from build123d import *

# Parameters (mm, degrees)
BASE_PLATE_140X70X20_DEPTH   = 20
CENTRE_HOLE_SKETCH_R         = 10
CENTRE_HOLE_20_DEPTH         = 20
CENTRE_POCKET_SKETCH_W       = 40
CENTRE_POCKET_SKETCH_H       = 40
CENTRE_POCKET_40X40X10_DEPTH = 10
V_BLOCK_UPRIGHTS_DEPTH       = 70
GUSSET_RIB_DEPTH             = 5


with BuildPart() as part:
    # Base Plate Sketch → Base Plate 140x70x20 (new body)
    with BuildSketch(Plane(origin=(0, 0, 0), x_dir=(1, 0, 0), z_dir=(0, 1, 0))):
        with BuildLine():
            Line((-70, 25), (-62.5, 25))
            ThreePointArc((-62.5, 25), (-57.5, 20), (-62.5, 15))
            Line((-62.5, 15), (-70, 15))
            Line((-70, 15), (-70, -15))
            Line((-70, -15), (-62.5, -15))
            ThreePointArc((-62.5, -15), (-57.5, -20), (-62.5, -25))
            Line((-62.5, -25), (-70, -25))
            Line((-70, -25), (-70, -35))
            Line((-70, -35), (70, -35))
            Line((70, -35), (70, -25))
            Line((70, -25), (62.5, -25))
            ThreePointArc((62.5, -25), (57.5, -20), (62.5, -15))
            Line((62.5, -15), (70, -15))
            Line((70, -15), (70, 15))
            Line((70, 15), (62.5, 15))
            ThreePointArc((62.5, 15), (57.5, 20), (62.5, 25))
            Line((62.5, 25), (70, 25))
            Line((70, 25), (70, 35))
            Line((70, 35), (-70, 35))
            Line((-70, 35), (-70, 25))
        make_face()
    extrude(amount=BASE_PLATE_140X70X20_DEPTH)

    # Centre Hole Sketch → Centre Hole Ø20 (cut)
    with BuildSketch(Plane(origin=(0, 20, 0), x_dir=(1, 0, 0), z_dir=(0, 1, 0))):
        with Locations(Location((0, 0, 0), (0, 0, 270))):
            Circle(CENTRE_HOLE_SKETCH_R)
    extrude(amount=-CENTRE_HOLE_20_DEPTH, mode=Mode.SUBTRACT)

    # Centre Pocket Sketch → Centre Pocket 40x40x10 (cut)
    with BuildSketch(Plane(origin=(0, 20, 0), x_dir=(1, 0, 0), z_dir=(0, 1, 0))):
        Rectangle(CENTRE_POCKET_SKETCH_W, CENTRE_POCKET_SKETCH_H)
    extrude(amount=-CENTRE_POCKET_40X40X10_DEPTH, mode=Mode.SUBTRACT)

    # V-Block Uprights Sketch → V-Block Uprights (add)
    with BuildSketch(Plane.XY.offset(35)):
        Polygon((-40, 60), (-52.5, 20), (-35, 20), (-35, 60), align=None)
        Polygon((35, 60), (35, 20), (52.5, 20), (40, 60), align=None)
    extrude(amount=-V_BLOCK_UPRIGHTS_DEPTH)

    # Gusset Rib Sketch → Gusset Rib (add, symmetric)
    with BuildSketch(Plane.XY):
        Polygon((-20.102951906, 20), (-35, 20), (-35, 52), align=None)
        Polygon((20.1, 20), (35, 52), (35, 20), align=None)
    extrude(amount=GUSSET_RIB_DEPTH, both=True)


solid = part.part
The listing builds one solid part. Answer for the finished solid, in the listing's coordinates (mm). A direction names the side the tool comes from. Round coordinates to 2 decimals unless told otherwise and drop trailing zeros. Order: outer loops, then holes, each group sorted by start corner. A loop starts at its lowest first (then second) coordinate and runs counter-clockwise, first axis right, second up. Notation, with made-up numbers: M 1.25,21.5 L 49.25,21.5 A8 ccw 49.25,28.5 Z; hole C -22,-35.5 d4. An arc over 180 degrees is marked long. Answer in a Markdown table with one row per item. Add a question column.
1) Flat-ended cylindrical pins translate along their axes: pin 1 Ø1 at (y, z) = (53.5, -7.5) entering from +X; pin 2 Ø12 at (y, z) = (52, -13.5) entering from +X (3 decimals); pin 3 Ø12 at (x, z) = (9, 0.5) entering from +Y. Find the tip coordinate at first contact, or state that the pin passes through.
2) The part is cut by section A-A on y = 4. Determine the outline of the cut face in (x, z), plus the area to 3 significant figures.
3) The part is cut by section B-B on x = 17.5. Determine the outline of the cut face in (y, z).
4) Determine the mould class of faces 4 (the face through (-57.5, 9.9, 19.9)), 5 (the face through (0, 15, 20)), 6 (the face through (20, 15, 0)), 7 (the face through (-66, 10, -25)) for opening direction X: pulls with the +X half, pulls with the -X half, needs draft (parallel to the pull), parting line crosses it, or undercut.
5) Which of the six approach directions +Z, -Z, +X, -X, +Y, -Y give full straight-line access (tool end or side, diameter ignored) to faces 1 (the face through (-5, 10, -9)), 2 (the face through (-59, 20, 0)), 3 (the face through (66, 10, -25))?
6) The part is cut by section D-D on x = 0. Determine the outline of the cut face in (y, z).
7) The part is cut by section C-C on z = 0. Determine the outline of the cut face in (x, y).
8) Consider line 1 along Z through (x, y) = (-62, 14); line 2 along X through (y, z) = (5, 0); line 3 along Y through (x, z) = (20.5, -6). Determine where each line is inside the solid, lowest interval first. Write a range as from..to.
Findings below:
| question | item | result |
|---|---|---|
| 1 | pin 1 | stops at x = 42.19 |
| 1 | pin 2 | stops at x = 44.375 |
| 1 | pin 3 | stops at y = 10 |
| 2 | outline | M -70,-35 L 70,-35 L 70,-25 L 62.5,-25 A5 cw 62.5,-15 L 70,-15 L 70,15 L 62.5,15 A5 cw 62.5,25 L 70,25 L 70,35 L -70,35 L -70,25 L -62.5,25 A5 cw -62.5,15 L -70,15 L -70,-15 L -62.5,-15 A5 cw -62.5,-25 L -70,-25 Z; hole C 0,0 d20 |
| 2 | area | 9,030 mm² |
| 3 | outline | M 0,-35 L 20,-35 L 20,-20 L 10,-20 L 10,20 L 20,20 L 20,35 L 0,35 Z |
| 4 | face 4 | pulls with the -X half |
| 4 | face 5 | undercut |
| 4 | face 6 | undercut |
| 4 | face 7 | needs draft |
| 5 | face 1 | +Y |
| 5 | face 2 | +Z, -Z, -X, +Y |
| 5 | face 3 | +X, +Y, -Y |
| 6 | outline | M 0,-35 L 20,-35 L 20,-20 L 10,-20 L 10,-10 L 0,-10 Z; M 0,10 L 10,10 L 10,20 L 20,20 L 20,35 L 0,35 Z |
| 7 | outline | M -70,0 L -10,0 L -10,10 L -20,10 L -20,20 L -20.1,20 L -35,52 L -35,60 L -40,60 L -52.5,20 L -70,20 Z; M 10,0 L 70,0 L 70,20 L 52.5,20 L 40,60 L 35,60 L 35,52 L 20.1,20 L 20,20 L 20,10 L 10,10 Z |
| 8 | line 1 | z = -35..-24.97, -15.03..15.03, 24.97..35 |
| 8 | line 2 | x = -70..-10, 10..70 |
| 8 | line 3 | y = 0..20 |
